```python
from build123d import *

# Parameters (mm, degrees)
SKETCH1_R           = 57.5
SKETCH1_R_2         = 9
BOSS_EXTRUDE1_DEPTH = 3.5


with BuildPart() as part:
    # Sketch1 → Boss-Extrude1 (new body)
    with BuildSketch(Plane.XY):
        with BuildLine():
            Line((-4.829629131, 129.527129815), (-10.18861298, 109.527129815))
            ThreePointArc((-10.18861298, 109.527129815), (0, -110), (10.18861298, 109.527129815))
            Line((10.18861298, 109.527129815), (4.829629131, 129.527129815))
            ThreePointArc((4.829629131, 129.527129815), (0, 133.23303459), (-4.829629131, 129.527129815))
        make_face()
        Circle(SKETCH1_R, mode=Mode.SUBTRACT)
        with Locations((0, 90)):
            Circle(SKETCH1_R_2, mode=Mode.SUBTRACT)
        with Locations((63.639610307, 63.639610307)):
            Circle(SKETCH1_R_2, mode=Mode.SUBTRACT)
        with Locations((90, 0)):
            Circle(SKETCH1_R_2, mode=Mode.SUBTRACT)
        with Locations((63.639610307, -63.639610307)):
            Circle(SKETCH1_R_2, mode=Mode.SUBTRACT)
        with Locations((0, -90)):
            Circle(SKETCH1_R_2, mode=Mode.SUBTRACT)
        with Locations((-63.639610307, -63.639610307)):
            Circle(SKETCH1_R_2, mode=Mode.SUBTRACT)
        with Locations((-90, 0)):
            Circle(SKETCH1_R_2, mode=Mode.SUBTRACT)
        with Locations((-63.639610307, 63.639610307)):
            Circle(SKETCH1_R_2, mode=Mode.SUBTRACT)
    extrude(amount=BOSS_EXTRUDE1_DEPTH)


solid = part.part
```
Could you check a few things on this model? Use its own coordinates, in mm. Round coordinates to 2 decimals unless told otherwise and drop trailing zeros. Loops run counter-clockwise (first coordinate to the right, second up) from the corner with the lowest first, then second, coordinate; pieces in that order, holes last. Notation, with made-up numbers: M 85,-24 L 132,-24 A8 cw 132,-15 Z; hole C -6,10 d2. An arc over 180 degrees is marked long. Write item = value, one per line.
1. I want a section at B-B, the plane x = 15.5. Write out the boundary of the cut face in (y, z), and give its area (3 significant figures).
Results below:
outline = M -108.9,0 L -55.37,0 L -55.37,3.5 L -108.9,3.5 Z; M 55.37,0 L 108.9,0 L 108.9,3.5 L 55.37,3.5 Z
area = 375 mm²
2. Will these pins go through, and if not, where does the flat tip stop? P1, Ø2, axis at y = 79.5, z = 1, coming from the -X side; P2, Ø2, axis at y = 13, z = 2.5, coming from the -X side; P3, Ø2, axis at x = -4.5, z = 2, coming from the +Y side.
Results below:
P1 = -77.06
P2 = -109.34
P3 = 131.8
3. I need wall thicknesses on probe 1 along Y at (x, z) = (0, 0.7); probe 2 along Y at (x, z) = (-62, 0.65); probe 3 along Y at (x, z) = (49.5, 2.35). Which ranges of each line are inside material? Lowest first, please.
Results below:
probe_1 = -110 to -99, -81 to -57.5, 57.5 to 81, 99 to 133.23
probe_2 = -90.86 to -72.49, -54.79 to 54.79, 72.49 to 90.86
probe_3 = -98.23 to -29.26, 29.26 to 98.23
4. I want a section at C-C, the plane x = -70. Write out the boundary of the cut face in (y, z).
Results below:
outline = M -84.85,0 L -70.01,0 L -70.01,3.5 L -84.85,3.5 Z; M -57.27,0 L 57.27,0 L 57.27,3.5 L -57.27,3.5 Z; M 70.01,0 L 84.85,0 L 84.85,3.5 L 70.01,3.5 Z
5. I want a section at A-A, the plane y = 0. Write out the boundary of the cut face in (x, z), and give its area (4 significant figures).
Results below:
outline = M -110,0 L -99,0 L -99,3.5 L -110,3.5 Z; M -81,0 L -57.5,0 L -57.5,3.5 L -81,3.5 Z; M 57.5,0 L 81,0 L 81,3.5 L 57.5,3.5 Z; M 99,0 L 110,0 L 110,3.5 L 99,3.5 Z
area = 241.5 mm²
6. I want a section at D-D, the plane y = -90. Write out the boundary of the cut face in (x, z), and give its area (3 significant figures).
Results below:
outline = M -63.25,0 L -9,0 L -9,3.5 L -63.25,3.5 Z; M 9,0 L 63.25,0 L 63.25,3.5 L 9,3.5 Z
area = 380 mm²
7. Thinking about a two-plate mould opening in X: for faces 1 (the face through (-81.416, 2.703, 1.726)), 2 (the face through (-72.63, -63.24, 1.73)), 3 (the face through (-4.7, -109.9, 1.7)), 4 (the face through (7.547, 119.387, 1.726)), which applies, +X half, -X half, draft (parallel to the pull), parting line (faces both ways), or undercut?
Results below:
face_1 = undercut
face_2 = undercut
face_3 = parting line
face_4 = +X half
